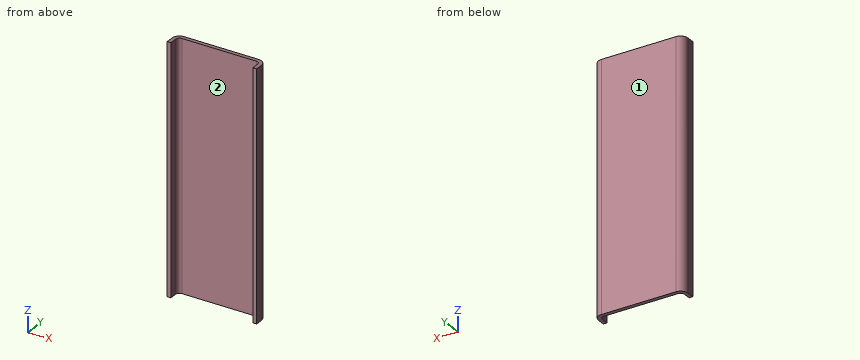
```python
from build123d import *

# Parameters (mm, degrees)
EXTRUDE_1_DEPTH = 320
EXTRUDE_START   = 10
EXTRUDE_2_DEPTH = 10


with BuildPart() as part:
    # 草图1 → 凸台-拉伸1 (new body)
    with BuildSketch(Plane.XY):
        with BuildLine():
            Line((10, 0), (110, 0))
            ThreePointArc((110, 0), (117.071067812, -2.928932188), (120, -10))
            Line((120, -10), (120, -20))
            Line((120, -20), (115, -20))
            Line((115, -20), (115, -10))
            ThreePointArc((115, -10), (113.535533906, -6.464466094), (110, -5))
            Line((110, -5), (10, -5))
            ThreePointArc((10, -5), (6.464466094, -6.464466094), (5, -10))
            Line((5, -10), (5, -20))
            Line((5, -20), (0, -20))
            Line((0, -20), (0, -10))
            ThreePointArc((0, -10), (2.928932188, -2.928932188), (10, 0))
        make_face()
    extrude(amount=EXTRUDE_1_DEPTH)

    # 草图2 → 凸台-拉伸2 (add)
    with BuildSketch(Plane(origin=(0, 0, 0), x_dir=(-1, 0, 0), z_dir=(0, 0, -1)).offset(EXTRUDE_START)):
        with BuildLine():
            Line((-120, -20), (-115, -20))
            Line((-115, -20), (-115, -10))
            ThreePointArc((-115, -10), (-113.535533906, -6.464466094), (-110, -5))
            Line((-110, -5), (-10, -5))
            ThreePointArc((-10, -5), (-6.464466094, -6.464466094), (-5, -10))
            Line((-5, -10), (-5, -20))
            Line((-5, -20), (0, -20))
            Line((0, -20), (0, -10))
            ThreePointArc((0, -10), (-2.928932188, -2.928932188), (-10, 0))
            Line((-10, 0), (-110, 0))
            ThreePointArc((-110, 0), (-117.071067812, -2.928932188), (-120, -10))
            Line((-120, -10), (-120, -20))
        make_face()
    extrude(amount=-EXTRUDE_2_DEPTH)


solid = part.part
```
Source: CAD feature listing. Evaluate the final solid. Frame: model axes, mm. Face numbers are marked on the shaded views. Round coordinates to 2 decimals unless told otherwise and drop trailing zeros. Write each loop counter-clockwise with the first axis right and the second up, starting at its lowest first coordinate (ties: lowest second). Pieces come first, ordered by that corner, then holes. Notation, with made-up numbers: M 4.5,57.5 L 20.5,57.5 A38 cw 20.5,95.5 Z; hole C 24.25,-12 d7. An arc over 180 degrees is marked long. Answer as a JSON object with one key per item and string values. Group by question number.
(1) Ray query, line 1 (X direction, y = -18.75, z = 104); line 2 (Y direction, x = 63, z = 249); line 3 (X direction, y = -5.75, z = 71.5). Return the intervals inside material, ascending. Write a range as [from, to].
(2) Mould query, pull axis X, two halves, no side actions, for the marked faces 1 and 2. Classes: +X half, -X half, draft (parallel to the pull), parting line (faces both ways), or undercut.
(3) Section query C-C on x = 22.5. Output: boundary loops of the cut face in (y, z), then the cut area to 3 significant figures.
(4) First-contact query: pin 1 (4 mm diameter, centred on y = -7, z = 97.5, fed in from -X); pin 2 (12 mm diameter, centred on x = 79.5, z = 145, fed in from -Y). Flat tips, straight axial feed; report the tip coordinate or a pass-through.
(5) Section query B-B on z = 39. Output: boundary loops of the cut face in (x, y).
(6) Section query A-A on y = -16. Output: boundary loops of the cut face in (x, z), then the cut area to 3 significant figures.
Computed values:
{
 "1": {"line 1": "[0, 5], [115, 120]", "line 2": "[-5, 0]", "line 3": "[0.95, 7.37], [112.63, 119.05]"},
 "2": {"face 1": "draft", "face 2": "undercut"},
 "3": {"outline": "M -5,-10 L 0,-10 L 0,320 L -5,320 Z", "area": "1,650 mm^2"},
 "4": {"pin 1": "x = 0.05", "pin 2": "y = -5"},
 "5": {"outline": "M 0,-20 L 5,-20 L 5,-10 A5 cw 10,-5 L 110,-5 A5 cw 115,-10 L 115,-20 L 120,-20 L 120,-10 A10 ccw 110,0 L 10,0 A10 ccw 0,-10 Z"},
 "6": {"outline": "M 0,-10 L 5,-10 L 5,320 L 0,320 Z; M 115,-10 L 120,-10 L 120,320 L 115,320 Z", "area": "3,300 mm^2"}
}
